The figure shows three views and two pictorial views of one solid part (mm, origin at its lowest corner). Answer the questions. Round coordinates to 2 decimals unless told otherwise and drop trailing zeros. Write each loop counter-clockwise with the first axis right and the second up, starting at its lowest first coordinate (ties: lowest second). Pieces come first, ordered by that corner, then holes.
Item 1: Find section D-D on y = 2.75. Give the vertices of the cut face in (x, z).
Item 2: Find section C-C on z = 15. Give the vertices of the cut face in (x, y).
Item 3: For a pull along Z with two mould halves and no side action, classify the marked faces 1, 2 and 3 as +Z half, -Z half, draft (parallel to the pull), parting line (faces both ways), or undercut.
Item 4: Find section A-A on x = 135. Give the vertices of the cut face in (y, z).
Item 5: Find the intervals of material crossed by probe 1 along X at (y, z) = (2, 15.25); probe 2 along Z at (x, y) = (15, 2.95); probe 3 along X at (y, z) = (1.5, 19), in increasing order.
Item 6: Find section B-B on y = 8.25. Give the vertices of the cut face in (x, z), then the cut area to 3 significant figures.
Item 7: This flat-tipped pin is pushed along its axis until it touches: pin 1 (10.5 mm diameter, centred on x = 135, z = 15, fed in from +Y). Where does it stop, or does it pass through?
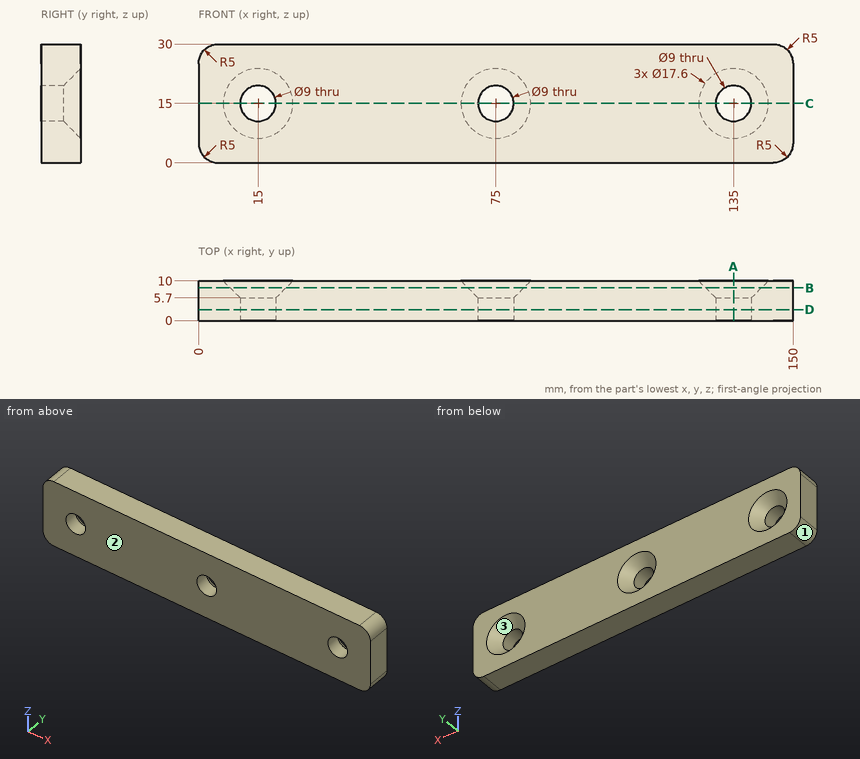
Check values:
1. outline: (0, 5) arc R5 ccw to (5, 0) - (145, 0) arc R5 ccw to (150, 5) - (150, 25) arc R5 ccw to (145, 30) - (5, 30) arc R5 ccw to (0, 25) - close; hole circle Ø9 at (15, 15); hole circle Ø9 at (75, 15); hole circle Ø9 at (135, 15)
2. outline: (0, 0) - (10.5, 0) - (10.5, 5.7) - (6.2, 10) - (0, 10) - close; (19.5, 0) - (70.5, 0) - (70.5, 5.7) - (66.2, 10) - (23.8, 10) - (19.5, 5.7) - close; (79.5, 0) - (130.5, 0) - (130.5, 5.7) - (126.2, 10) - (83.8, 10) - (79.5, 5.7) - close; (139.5, 0) - (150, 0) - (150, 10) - (143.8, 10) - (139.5, 5.7) - close
3. face 1: -Z half
3. face 2: draft
3. face 3: undercut
4. outline: (0, 0) - (10, 0) - (10, 6.2) - (5.7, 10.5) - (0, 10.5) - close; (0, 19.5) - (5.7, 19.5) - (10, 23.8) - (10, 30) - (0, 30) - close
5. probe 1: x = 0 to 10.51, 19.49 to 70.51, 79.49 to 130.51, 139.49 to 150
5. probe 2: z = 0 to 10.5, 19.5 to 30
5. probe 3: x = 0 to 12.94, 17.06 to 72.94, 77.06 to 132.94, 137.06 to 150
6. outline: (0, 5) arc R5 ccw to (5, 0) - (145, 0) arc R5 ccw to (150, 5) - (150, 25) arc R5 ccw to (145, 30) - (5, 30) arc R5 ccw to (0, 25) - close; hole circle Ø14.1 at (15, 15); hole circle Ø14.1 at (75, 15); hole circle Ø14.1 at (135, 15)
6. area: 4,010 mm2
7. pin 1: stops at y = 6.45
